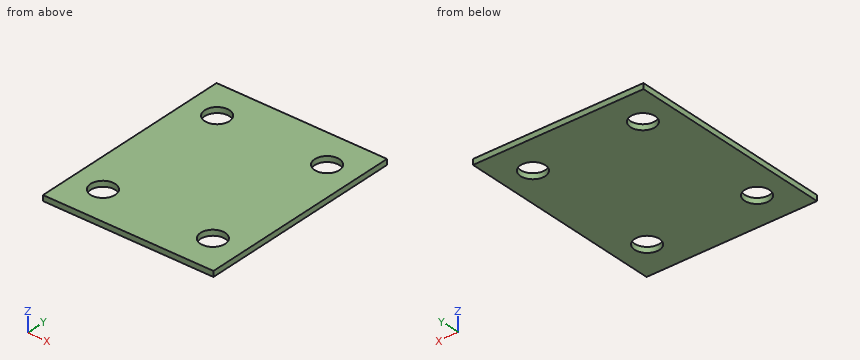
from build123d import *

# Parameters (mm, degrees)
SKETCH_1_W      = 31
SKETCH_1_H      = 38
SKETCH_1_R      = 2.25
EXTRUDE_1_DEPTH = 1


with BuildPart() as part:
    # 草图1 → 凸台-拉伸1 (new body)
    with BuildSketch(Plane.XY):
        Rectangle(SKETCH_1_W, SKETCH_1_H)
        with Locations((-10, 12.5)):
            Circle(SKETCH_1_R, mode=Mode.SUBTRACT)
        with Locations((10, 12.5)):
            Circle(SKETCH_1_R, mode=Mode.SUBTRACT)
        with Locations((10, -12.5)):
            Circle(SKETCH_1_R, mode=Mode.SUBTRACT)
        with Locations((-10, -12.5)):
            Circle(SKETCH_1_R, mode=Mode.SUBTRACT)
    extrude(amount=EXTRUDE_1_DEPTH)


solid = part.part
Verification items for the finished model (mm, model axes). Coordinates: 2 decimals unless noted, no trailing zeros. Write each loop counter-clockwise with the first axis right and the second up, starting at its lowest first coordinate (ties: lowest second). Pieces come first, ordered by that corner, then holes. Notation, with made-up numbers: M -13,75 L 46,75 A18 ccw 46,100 Z; hole C -11.5,-27.5 d7. An arc over 180 degrees is marked long. Use CSV: the item, a comma, the result in double quotes.
Q1. Thickness scan on line 1 along Y through (x, z) = (-10, 0.25); line 2 along Y through (x, z) = (-8, 0.9); line 3 along X through (y, z) = (-11.5, 0.6). Record the ranges inside material, lowest first. Write a range as [from, to].
Computed values:
line 1,"[-19, -14.75], [-10.25, 10.25], [14.75, 19]"
line 2,"[-19, -13.53], [-11.47, 11.47], [13.53, 19]"
line 3,"[-15.5, -12.02], [-7.98, 7.98], [12.02, 15.5]"
Q2. Go/stop test with a flat-tipped pin: P1, Ø3.5, axis at x = 10, y = 12.5, coming from the -Z side. Record where the tip stops, or that it passes through.
Computed values:
P1,"through"
Q3. Section check C-C, the plane y = 11.5. Enter the section's corners in (x, z), and give its area (3 significant figures).
Computed values:
outline,"M -15.5,0 L -12.02,0 L -12.02,1 L -15.5,1 Z; M -7.98,0 L 7.98,0 L 7.98,1 L -7.98,1 Z; M 12.02,0 L 15.5,0 L 15.5,1 L 12.02,1 Z"
area,"22.9 mm²"
Q4. Section check B-B, the plane z = 0.25. Enter the section's corners in (x, y), and give its area (3 significant figures).
Computed values:
outline,"M -15.5,-19 L 15.5,-19 L 15.5,19 L -15.5,19 Z; hole C -10,-12.5 d4.5; hole C -10,12.5 d4.5; hole C 10,-12.5 d4.5; hole C 10,12.5 d4.5"
area,"1,110 mm²"
Q5. Section check A-A, the plane x = -10. Enter the section's corners in (y, z).
Computed values:
outline,"M -19,0 L -14.75,0 L -14.75,1 L -19,1 Z; M -10.25,0 L 10.25,0 L 10.25,1 L -10.25,1 Z; M 14.75,0 L 19,0 L 19,1 L 14.75,1 Z"
